Source: CAD feature listing. Evaluate the final solid. Frame: model axes, mm. A direction names the side the tool comes from. Give positions to 0.01 mm unless a question says otherwise; leave off trailing zeros. Write each loop counter-clockwise with the first axis right and the second up, starting at its lowest first coordinate (ties: lowest second). Pieces come first, ordered by that corner, then holes. Notation, with made-up numbers: (13, 34.5) -> (67, 34.5) arc R34 cw to (67, 71.5) -> close; hole circle Ø4 at (26, 72.5). An arc over 180 degrees is marked (long way). Use one line per item in the form item = value. Start each with the question number.
(1) Cut plane C-C, the plane z = 14. Output: boundary loops of the cut face in (x, y).
(2) First-contact query: P1, Ø2, axis at x = 32, z = 21, coming from the -Y side; P2, Ø15.5, axis at x = 86.5, z = 11.5, coming from the -Y side; P3, Ø6, axis at y = -20.5, z = 22.5, coming from the -X side; P4, Ø7, axis at x = 65, z = 14, coming from the +Y side (1 decimal). Flat tips, straight axial feed; report the tip coordinate or a pass-through.
(3) Material intervals for line 1 along Y through (x, z) = (89.5, 14); line 2 along X through (y, z) = (-17, 14); line 3 along X through (y, z) = (-1, 11.75), sorted ascending. Write a range as from..to.
(4) Draft query along X for faces 1 (the face through (95, -18, 17)), 2 (the face through (88, -35, 14)), 3 (the face through (81, -19, 14)). Return one class per face: pulls with the +X half, pulls with the -X half, needs draft (parallel to the pull), parting line crosses it, or undercut.
(5) Set-up query: faces 4 (the face through (88.098, -10.698, 8.277)), 5 (the face through (60, 1, 0)), 6 (the face through (80.1, -0.86, 13.8)). Return all of +Z, -Z, +X, -X, +Y, -Y with unobstructed straight access to the full face (end or side cutting, diameter ignored); none if empty.
(6) Cut plane B-B, the plane y = -12.5. Output: boundary loops of the cut face in (x, z), and give its area (3 significant figures).
(7) Cut plane D-D, the plane x = 83. Output: boundary loops of the cut face in (y, z), and give its area (3 significant figures).
(8) Cut plane A-A, the plane x = 0. Output: boundary loops of the cut face in (y, z).
from build123d import *

# Parameters (mm, degrees)
CRANK_ARM_DEPTH        = 28
PIVOT_HUB_DEPTH        = 21
PIVOT_HUB_DEPTH_BACK   = 46
PIVOT_HUB_SKETCH_R     = 15
PIVOT_HUB_SKETCH_R_2   = 7
HUB_FILLET_R1_R        = 1
TOP_START              = 132
TOP_THROUGH_HOLE_DEPTH = 132
ARM_HOLE_SKETCH_R      = 6
ARM_THROUGH_HOLE_DEPTH = 132
BORE_SKETCH_R          = 6
THROUGH_BORE_DEPTH     = 42


with BuildPart() as part:
    # Arm Profile Sketch → Crank Arm (new body)
    with BuildSketch(Plane.XY):
        with BuildLine():
            Line((0, 0), (78, 0))
            ThreePointArc((78, 0), (80.121320344, -0.878679656), (81, -3))
            Line((81, -3), (81, -35))
            Line((81, -35), (95, -35))
            Line((95, -35), (95, 10))
            Line((95, 10), (0, 10))
            Line((0, 10), (0, 0))
        make_face()
    extrude(amount=CRANK_ARM_DEPTH)

    # Pivot Hub Sketch → Pivot Hub (add, two sides: drawn at the far end of the back side and taken through both)
    with BuildSketch(Plane(origin=(0, 10, 0), x_dir=(1, 0, 0), z_dir=(0, 1, 0)).offset(-PIVOT_HUB_DEPTH_BACK)):
        with Locations(Location((0, -14, 0), (0, 0, 270))):
            Circle(PIVOT_HUB_SKETCH_R)
        with Locations(Location((0, -14, 0), (0, 0, 270))):
            Circle(PIVOT_HUB_SKETCH_R_2, mode=Mode.SUBTRACT)
    extrude(amount=PIVOT_HUB_DEPTH + PIVOT_HUB_DEPTH_BACK)

    # Hub Fillet R1
    hub_fillet_r1_edges = [part.edges().sort_by_distance(p)[0] for p in [
        (5.385164807, 5, 0),
        (5.385164807, 5, 28),
    ]]
    fillet(hub_fillet_r1_edges, radius=HUB_FILLET_R1_R)

    # Top Hole Sketch → Top Through Hole (cut)
    with BuildSketch(Plane(origin=(0, 0, 0), x_dir=(1, 0, 0), z_dir=(0, 1, 0)).offset(TOP_START)):
        with BuildLine():
            Line((0, -7), (0, -21))
            ThreePointArc((0, -21), (7, -14), (0, -7))
        make_face()
    extrude(amount=-TOP_THROUGH_HOLE_DEPTH, mode=Mode.SUBTRACT)

    # Arm Hole Sketch → Arm Through Hole (cut)
    with BuildSketch(Plane(origin=(0, 10, 0), x_dir=(1, 0, 0), z_dir=(0, 1, 0))):
        with Locations(Location((65, -14, 0), (0, 0, 270))):
            Circle(ARM_HOLE_SKETCH_R)
    extrude(amount=-ARM_THROUGH_HOLE_DEPTH, mode=Mode.SUBTRACT)

    # Bore Sketch → Through Bore (cut)
    with BuildSketch(Plane(origin=(95, 0, 0), x_dir=(0, 0, -1), z_dir=(1, 0, 0))):
        with Locations((-14, -12.5)):
            Circle(BORE_SKETCH_R)
    extrude(amount=-THROUGH_BORE_DEPTH, mode=Mode.SUBTRACT)


solid = part.part
Geometry says:
q1.outline = (-15, -36) -> (-7, -36) -> (-7, 31) -> (-15, 31) -> close; (7, -36) -> (15, -36) -> (15, 0) -> (59, 0) -> (59, 10) -> (15, 10) -> (15, 31) -> (7, 31) -> close; (71, 0) -> (78, 0) arc R3 cw to (81, -3) -> (81, -6.5) -> (95, -6.5) -> (95, 10) -> (71, 10) -> close; (81, -35) -> (95, -35) -> (95, -18.5) -> (81, -18.5) -> close
q2.P1 = 0
q2.P2 = -35
q2.P3 = -13.96
q2.P4 = through
q3.line_1 = -35..-18.5, -6.5..10
q3.line_2 = -15..-7, 7..15
q3.line_3 = -14.83..-6.63, 6.63..14.83, 80.24..95
q4.face_1 = pulls with the +X half
q4.face_2 = needs draft
q4.face_3 = undercut
q5.face_4 = +X
q5.face_5 = -Z, +X, +Y, -Y
q5.face_6 = +Z, -Z, -Y
q6.outline = circle Ø30 at (0, 14); (81, 0) -> (95, 0) -> (95, 8) -> (81, 8) -> close; (81, 20) -> (95, 20) -> (95, 28) -> (81, 28) -> close; hole circle Ø14 at (0, 14)
q6.area = 777 mm^2
q7.outline = (-35, 0) -> (10, 0) -> (10, 28) -> (-35, 28) -> close; hole circle Ø12 at (-12.5, 14)
q7.area = 1,150 mm^2
q8.outline = (-36, -1) -> (31, -1) -> (31, 7) -> (-36, 7) -> close; (-36, 21) -> (31, 21) -> (31, 29) -> (-36, 29) -> close
